from build123d import *

# Parameters (mm, degrees)
BOSS_EXTRUDE1_DEPTH   = 35
FILLET1_R             = 3
M8X1_0_TAPPED_HOLE1_D = 7
CUT_EXTRUDE1_DEPTH    = 43.577310513
CUT_EXTRUDE2_DEPTH    = 4.5


with BuildPart() as part:
    # Sketch1 → Boss-Extrude1 (new body)
    with BuildSketch(Plane(origin=(0, 0, 0), x_dir=(1, 0, 0), z_dir=(0, 1, 0))):
        with BuildLine():
            Line((-22.5, 81.967981554), (-22.5, 91))
            Line((-22.5, 91), (22.5, 91))
            Line((22.5, 91), (22.5, 81.967981554))
            ThreePointArc((22.5, 81.967981554), (0, 85), (-22.5, 81.967981554))
        make_face()
    extrude(amount=BOSS_EXTRUDE1_DEPTH)

    # Fillet1
    fillet1_edges = [part.edges().sort_by_distance(p)[0] for p in [
        (22.5, 35, -86.483990777),
        (22.5, 0, -86.483990777),
        (-22.5, 0, -86.483990777),
        (-22.5, 35, -86.483990777),
    ]]
    fillet(fillet1_edges, radius=FILLET1_R)

    # M8x1.0 Tapped Hole1 (through all)
    with Locations(Plane(origin=(0, 0, -91), x_dir=(-1, 0, 0), z_dir=(0, 0, -1))):
        with Locations((0, 17.5)):
            Hole(M8X1_0_TAPPED_HOLE1_D / 2)

    # Sketch4 → Cut-Extrude1 (cut, through all)
    with BuildSketch(Plane(origin=(0, 0, -91), x_dir=(-1, 0, 0), z_dir=(0, 0, -1))):
        with BuildLine():
            Line((-12.25, 30), (-12.25, 5))
            ThreePointArc((-12.25, 5), (-14.5, 2.75), (-16.75, 5))
            Line((-16.75, 5), (-16.75, 30))
            ThreePointArc((-16.75, 30), (-14.5, 32.25), (-12.25, 30))
        make_face()
        with BuildLine():
            Line((16.75, 30), (16.75, 5))
            ThreePointArc((16.75, 5), (14.5, 2.75), (12.25, 5))
            Line((12.25, 5), (12.25, 30))
            ThreePointArc((12.25, 30), (14.5, 32.25), (16.75, 30))
        make_face()
    extrude(amount=-CUT_EXTRUDE1_DEPTH, mode=Mode.SUBTRACT)

    # Sketch5 → Cut-Extrude2 (cut)
    with BuildSketch(Plane(origin=(0, 0, -91), x_dir=(-1, 0, 0), z_dir=(0, 0, -1))):
        with BuildLine():
            Line((-10.5, 30), (-10.5, 5))
            ThreePointArc((-10.5, 5), (-14.5, 1), (-18.5, 5))
            Line((-18.5, 5), (-18.5, 30))
            ThreePointArc((-18.5, 30), (-14.5, 34), (-10.5, 30))
        make_face()
        with BuildLine():
            Line((18.5, 30), (18.5, 5))
            ThreePointArc((18.5, 5), (14.5, 1), (10.5, 5))
            Line((10.5, 5), (10.5, 30))
            ThreePointArc((10.5, 30), (14.5, 34), (18.5, 30))
        make_face()
    extrude(amount=-CUT_EXTRUDE2_DEPTH, mode=Mode.SUBTRACT)


solid = part.part
Geometry check sheet. Reference: the model listing, model coordinates, mm. A direction names the side the tool comes from. Give positions to 0.01 mm unless a question says otherwise; leave off trailing zeros. Order: outer loops, then holes, each group sorted by start corner. A loop starts at its lowest first (then second) coordinate and runs counter-clockwise, first axis right, second up. Notation, with made-up numbers: (70, 57.5) - (120, 57.5) arc R25 ccw to (120, 87.5) - close; hole circle Ø7 at (16.5, -40). An arc over 180 degrees is marked (long way). Use one line per item in the form item = value.
1) Sectioned sample at C-C (z = -88.75). Record the boundary of the cut face in (x, y), and give its area (3 significant figures).
Working result:
outline = (-22.5, 3) arc R3 ccw to (-19.5, 0) - (19.5, 0) arc R3 ccw to (22.5, 3) - (22.5, 32) arc R3 ccw to (19.5, 35) - (-19.5, 35) arc R3 ccw to (-22.5, 32) - close; hole (-18.5, 5) arc R4 ccw to (-10.5, 5) - (-10.5, 30) arc R4 ccw to (-18.5, 30) - close; hole circle Ø7 at (0, 17.5); hole (10.5, 5) arc R4 ccw to (18.5, 5) - (18.5, 30) arc R4 ccw to (10.5, 30) - close
area = 1,030 mm^2
2) Access from +Z, -Z, +X, -X, +Y, -Y to the whole of each face (thin tool, end or side, straight path). Record for faces 1 (the face through (14.6, 34, -88.8)), 2 (the face through (-0.31, 21.14, -91)), 3 (the face through (-16.75, 18, -85)).
Working result:
face_1 = -Z
face_2 = -Z, +X, -X, +Y, -Y
face_3 = +Z, -Z
3) Sectioned sample at B-B (y = 17.5). Record the boundary of the cut face in (x, z).
Working result:
outline = (-22.5, -91) - (-18.5, -91) - (-18.5, -86.5) - (-16.75, -86.5) - (-16.75, -83.33) arc R85 cw to (-22.5, -81.97) - close; (-12.25, -86.5) - (-10.5, -86.5) - (-10.5, -91) - (-3.5, -91) - (-3.5, -84.93) arc R85 cw to (-12.25, -84.11) - close; (3.5, -91) - (10.5, -91) - (10.5, -86.5) - (12.25, -86.5) - (12.25, -84.11) arc R85 cw to (3.5, -84.93) - close; (16.75, -86.5) - (18.5, -86.5) - (18.5, -91) - (22.5, -91) - (22.5, -81.97) arc R85 cw to (16.75, -83.33) - close
4) Sectioned sample at D-D (y = 8). Record the boundary of the cut face in (x, z), and give its area (3 significant figures).
Working result:
outline = (-22.5, -91) - (-18.5, -91) - (-18.5, -86.5) - (-16.75, -86.5) - (-16.75, -83.33) arc R85 cw to (-22.5, -81.97) - close; (-12.25, -86.5) - (-10.5, -86.5) - (-10.5, -91) - (10.5, -91) - (10.5, -86.5) - (12.25, -86.5) - (12.25, -84.11) arc R85 cw to (-12.25, -84.11) - close; (16.75, -86.5) - (18.5, -86.5) - (18.5, -91) - (22.5, -91) - (22.5, -81.97) arc R85 cw to (16.75, -83.33) - close
area = 218 mm^2
5) Material ranges on probe 1 along X at (y, z) = (17.5, -86.25); probe 2 along X at (y, z) = (17.5, -88); probe 3 along X at (y, z) = (24, -85.5), recorded low to high. Write a range as from..to.
Working result:
probe_1 = -22.5..-16.75, -12.25..-3.5, 3.5..12.25, 16.75..22.5
probe_2 = -22.5..-18.5, -10.5..-3.5, 3.5..10.5, 18.5..22.5
probe_3 = -22.5..-16.75, -12.25..12.25, 16.75..22.5
6) Depth check by flat-ended pin: pin 1 Ø5 at (x, z) = (2.5, -83) entering from -Y; pin 2 Ø3 at (x, y) = (8.5, 12.5) entering from +Z. Enter the tip coordinate at first touch or a pass-through.
Working result:
pin_1 = 0
pin_2 = -84.41
7) Sectioned sample at A-A (x = 0). Record the boundary of the cut face in (y, z).
Working result:
outline = (0, -91) - (14, -91) - (14, -85) - (0, -85) - close; (21, -91) - (35, -91) - (35, -85) - (21, -85) - close
